```python
from build123d import *

# Parameters (mm, degrees)
SKETCH1_R           = 283
SKETCH1_R_2         = 70
SKETCH1_R_3         = 15
SKETCH1_R_4         = 8
BOSS_EXTRUDE1_DEPTH = 12


with BuildPart() as part:
    # Sketch1 → Boss-Extrude1 (new body)
    with BuildSketch(Plane(origin=(0, 0, 0), x_dir=(1, 0, 0), z_dir=(0, 1, 0))):
        with Locations(Location((0, 0, 0), (0, 0, 270))):
            Circle(SKETCH1_R)
        with Locations(Location((0, 0, 0), (0, 0, 270))):
            Circle(SKETCH1_R_2, mode=Mode.SUBTRACT)
        with Locations(Location((0, 116, 0), (0, 0, 270))):
            Circle(SKETCH1_R_3, mode=Mode.SUBTRACT)
        with Locations(Location((0, 164, 0), (0, 0, 270))):
            Circle(SKETCH1_R_4, mode=Mode.SUBTRACT)
        with Locations(Location((56.091303505, 154.109589809, 0), (0, 0, 270))):
            Circle(SKETCH1_R_4, mode=Mode.SUBTRACT)
        with Locations(Location((105.417167989, 125.631288672, 0), (0, 0, 270))):
            Circle(SKETCH1_R_4, mode=Mode.SUBTRACT)
        with Locations(Location((142.028166221, 82, 0), (0, 0, 270))):
            Circle(SKETCH1_R_4, mode=Mode.SUBTRACT)
        with Locations(Location((161.508471494, 28.478301137, 0), (0, 0, 270))):
            Circle(SKETCH1_R_4, mode=Mode.SUBTRACT)
        with Locations(Location((161.508471494, -28.478301137, 0), (0, 0, 270))):
            Circle(SKETCH1_R_4, mode=Mode.SUBTRACT)
        with Locations(Location((142.028166221, -82, 0), (0, 0, 270))):
            Circle(SKETCH1_R_4, mode=Mode.SUBTRACT)
        with Locations(Location((105.417167989, -125.631288672, 0), (0, 0, 270))):
            Circle(SKETCH1_R_4, mode=Mode.SUBTRACT)
        with Locations(Location((56.091303505, -154.109589809, 0), (0, 0, 270))):
            Circle(SKETCH1_R_4, mode=Mode.SUBTRACT)
        with Locations(Location((0, -164, 0), (0, 0, 270))):
            Circle(SKETCH1_R_4, mode=Mode.SUBTRACT)
        with Locations(Location((-56.091303505, -154.109589809, 0), (0, 0, 270))):
            Circle(SKETCH1_R_4, mode=Mode.SUBTRACT)
        with Locations(Location((-105.417167989, -125.631288672, 0), (0, 0, 270))):
            Circle(SKETCH1_R_4, mode=Mode.SUBTRACT)
        with Locations(Location((-142.028166221, -82, 0), (0, 0, 270))):
            Circle(SKETCH1_R_4, mode=Mode.SUBTRACT)
        with Locations(Location((-161.508471494, -28.478301137, 0), (0, 0, 270))):
            Circle(SKETCH1_R_4, mode=Mode.SUBTRACT)
        with Locations(Location((-161.508471494, 28.478301137, 0), (0, 0, 270))):
            Circle(SKETCH1_R_4, mode=Mode.SUBTRACT)
        with Locations(Location((-142.028166221, 82, 0), (0, 0, 270))):
            Circle(SKETCH1_R_4, mode=Mode.SUBTRACT)
        with Locations(Location((-105.417167989, 125.631288672, 0), (0, 0, 270))):
            Circle(SKETCH1_R_4, mode=Mode.SUBTRACT)
        with Locations(Location((-56.091303505, 154.109589809, 0), (0, 0, 270))):
            Circle(SKETCH1_R_4, mode=Mode.SUBTRACT)
        with Locations(Location((116, 0, 0), (0, 0, 270))):
            Circle(SKETCH1_R_3, mode=Mode.SUBTRACT)
        with Locations(Location((0, -116, 0), (0, 0, 270))):
            Circle(SKETCH1_R_3, mode=Mode.SUBTRACT)
        with Locations(Location((-116, 0, 0), (0, 0, 270))):
            Circle(SKETCH1_R_3, mode=Mode.SUBTRACT)
    extrude(amount=BOSS_EXTRUDE1_DEPTH)


solid = part.part
```
Here's how the part is built. I have some questions about the finished solid (model axes, mm). Coordinates: 2 decimals unless noted, no trailing zeros. Write each loop counter-clockwise with the first axis right and the second up, starting at its lowest first coordinate (ties: lowest second). Pieces come first, ordered by that corner, then holes. Notation, with made-up numbers: (-14, 61) - (-10, 61) arc R22 cw to (-10, 99) - close; hole circle Ø10 at (88.5, 58). An arc over 180 degrees is marked (long way). One line per item, written item: value.
1) We'd pull the mould along Z, two halves only. Please class faces 1 (the cylindrical face through (134.218, 5.916, 80.266)), 2 (the cylindrical face through (85.01, 5.92, 269.93)), 3 (the flat face through (-59, 0, 59)): pulls with the +Z half, pulls with the -Z half, needs draft (parallel to the pull), parting line crosses it, or undercut.
Model answer:
face 1: undercut
face 2: parting line crosses it
face 3: needs draft
2) Suppose I cut it at D-D on x = 233. Write out the boundary of the cut face in (y, z), and give its area (3 significant figures).
Model answer:
outline: (0, -160.62) - (12, -160.62) - (12, 160.62) - (0, 160.62) - close
area: 3,850 mm²
3) I need wall thicknesses on line 1 along X through (y, z) = (1.25, -85.5); line 2 along Z through (x, y) = (9.5, 4.25); line 3 along X through (y, z) = (10.75, -10). Which ranges of each line are inside material? Lowest first, please.
Model answer:
line 1: x = -269.78 to -149.22, -134.83 to 134.83, 149.22 to 269.78
line 2: z = -282.84 to -127.61, -104.39 to -69.35, 69.35 to 104.39, 127.61 to 282.84
line 3: x = -282.82 to -127.18, -104.82 to -69.28, 69.28 to 104.82, 127.18 to 282.82
4) Suppose I cut it at B-B on y = 5. State how many separate pieces and enclosed holes the cut face has, and give its area (3 significant figures).
Model answer:
separate pieces: 1
enclosed holes: 23
area: 230,000 mm²
5) Suppose I cut it at A-A on z = 0. Write out the boundary of the cut face in (x, y), and give its area (3 significant figures).
Model answer:
outline: (-283, 0) - (-131, 0) - (-131, 12) - (-283, 12) - close; (-101, 0) - (-70, 0) - (-70, 12) - (-101, 12) - close; (70, 0) - (101, 0) - (101, 12) - (70, 12) - close; (131, 0) - (283, 0) - (283, 12) - (131, 12) - close
area: 4,390 mm²
6) Suppose I cut it at C-C on z = -82. Write out the boundary of the cut face in (x, y), and give its area (3 significant figures).
Model answer:
outline: (-270.86, 0) - (-150.03, 0) - (-150.03, 12) - (-270.86, 12) - close; (-134.03, 0) - (134.03, 0) - (134.03, 12) - (-134.03, 12) - close; (150.03, 0) - (270.86, 0) - (270.86, 12) - (150.03, 12) - close
area: 6,120 mm²
7) I'm going to push flat-ended pins straight in: P1, Ø3, axis at y = 5, z = -212.5, coming from the -X side; P2, Ø1, axis at x = -219.5, y = 8, coming from the +Z side. Where does each tip first touch, or does it pass through?
Model answer:
P1: stops at x = -188.59
P2: stops at z = 179.24
